Geometry check sheet. Reference: the model listing, model coordinates, mm. A direction names the side the tool comes from. Round coordinates to 2 decimals unless told otherwise and drop trailing zeros. Write each loop counter-clockwise with the first axis right and the second up, starting at its lowest first coordinate (ties: lowest second). Pieces come first, ordered by that corner, then holes. Notation, with made-up numbers: (27, 79) - (41, 79) arc R26 cw to (41, 99) - close; hole circle Ø9 at (-12.5, 47.5). An arc over 180 degrees is marked (long way). Return JSON: item names as keys, results as strings.
```python
from build123d import *

# Parameters (mm, degrees)
BODY_PROFILE_SKETCH_R       = 3
PUMP_BODY_40MM_DEPTH        = 40
BODY_EDGE_FILLET_R8_R       = 8
CSK_HOLE_10_D               = 10
CSK_HOLE_10_CSINK_D         = 12
CSK_HOLE_10_CSINK_ANGLE     = 82
MOUNTING_FLANGE_10MM_DEPTH  = 10
FLANGE_RELIEF_CUT_REACH     = 90.436
FLANGE_RELIEF_CUT_SKETCH_R  = 8
CBORE_HOLE_6_D              = 6
CBORE_HOLE_6_CBORE_D        = 10
CBORE_HOLE_6_CBORE_DEPTH    = 5
SKETCH16_W                  = 3
SKETCH16_H                  = 10
PLAIN_HOLE_6_X10_AT_2_COUNT = 2
PLAIN_HOLE_6_X10_AT_2_PITCH = 80
LOCATING_BOSS_SKETCH_R      = 6
LOCATING_BOSS_12MM_DEPTH    = 12


with BuildPart() as part:
    # Body Profile Sketch → Pump Body 40mm (new body)
    with BuildSketch(Plane(origin=(0, 0, 0), x_dir=(0, 0, -1), z_dir=(1, 0, 0))):
        with BuildLine():
            Line((-12.5, -15.288884851), (-12.5, -36))
            ThreePointArc((-12.5, -36), (-12.104388127, -39.213597032), (-10.941176471, -42.235294118))
            ThreePointArc((-10.941176471, -42.235294118), (-11.140056594, -50.115966043), (-18, -54))
            Line((-18, -54), (-35, -54))
            Line((-35, -54), (-35, -64))
            Line((-35, -64), (35, -64))
            Line((35, -64), (35, -54))
            Line((35, -54), (18, -54))
            ThreePointArc((18, -54), (11.140056594, -50.115966043), (10.941176471, -42.235294118))
            ThreePointArc((10.941176471, -42.235294118), (12.104388127, -39.213597032), (12.5, -36))
            Line((12.5, -36), (12.5, -15.288884851))
            ThreePointArc((12.5, -15.288884851), (12.854205105, -13.25787525), (13.875, -11.466663639))
            ThreePointArc((13.875, -11.466663639), (17.99141486, -0.555869896), (14.556416913, 10.588235294))
            Line((14.556416913, 10.588235294), (6.469518628, 21.705882353))
            ThreePointArc((6.469518628, 21.705882353), (0, 25), (-6.469518628, 21.705882353))
            Line((-6.469518628, 21.705882353), (-14.556416913, 10.588235294))
            ThreePointArc((-14.556416913, 10.588235294), (-17.99141486, -0.555869896), (-13.875, -11.466663639))
            ThreePointArc((-13.875, -11.466663639), (-12.854205105, -13.25787525), (-12.5, -15.288884851))
        make_face()
        with Locations((0, -18)):
            Circle(BODY_PROFILE_SKETCH_R, mode=Mode.SUBTRACT)
        with Locations((0, 18)):
            Circle(BODY_PROFILE_SKETCH_R, mode=Mode.SUBTRACT)
    extrude(amount=PUMP_BODY_40MM_DEPTH)

    # Body Edge Fillet R8
    body_edge_fillet_r8_edges = [part.edges().sort_by_distance(p)[0] for p in [
        (0, -59, -35),
        (0, -59, 35),
        (40, -59, 35),
        (40, -59, -35),
    ]]
    fillet(body_edge_fillet_r8_edges, radius=BODY_EDGE_FILLET_R8_R)

    # Csk Hole Ø10 (through all)
    with Locations(Plane(origin=(10, -54, 27), x_dir=(0, 0, 1), z_dir=(0, 1, 0))):
        with Locations((0, 0), (0, 20)):
            csk_hole_10 = CounterSinkHole(CSK_HOLE_10_D / 2, CSK_HOLE_10_CSINK_D / 2, counter_sink_angle=CSK_HOLE_10_CSINK_ANGLE)

    # Csk Hole Ø10 Mirror: Csk Hole Ø10 across plane
    add(csk_hole_10.mirror(Plane.XY), mode=Mode.SUBTRACT)

    # Sketch7 → Main Bore Ø20 Csk Both Ends (revolve, cut)
    with BuildSketch(Plane(origin=(40, 0, 0), x_dir=(0, 0, -1), z_dir=(0, 1, 0))):
        Polygon((0, 0), (0, 40), (12, 40), (10, 37.699263186), (10, 2.300736814), (12, 0), align=None)
    revolve(axis=Axis((46.35, 0, 0), (-1, 0, 0)), mode=Mode.SUBTRACT)

    # Mounting Flange Sketch → Mounting Flange 10mm (add)
    with BuildSketch(Plane.ZY):
        with BuildLine():
            Line((32, 0), (32, -30))
            ThreePointArc((32, -30), (0, -62), (-32, -30))
            Line((-32, -30), (-32, 0))
            ThreePointArc((-32, 0), (0, 32), (32, 0))
        make_face()
    extrude(amount=MOUNTING_FLANGE_10MM_DEPTH)

    # Flange Relief Cut Sketch → Flange Relief Cut (cut, up to next)
    with BuildSketch(Plane.ZY.offset(10), mode=Mode.PRIVATE) as flange_relief_cut_sk1:
        Circle(FLANGE_RELIEF_CUT_SKETCH_R)
    flange_relief_cut_tool1 = extrude(flange_relief_cut_sk1.sketch, amount=-FLANGE_RELIEF_CUT_REACH, mode=Mode.PRIVATE) & part.part
    add(flange_relief_cut_tool1.solids().sort_by_distance((-10, 0, 0))[0], mode=Mode.SUBTRACT)

    # Sketch9 → Flange Csk Hole Ø18 (revolve, cut)
    with BuildSketch(Plane(origin=(-10, -36, 0), x_dir=(0, 0, 1), z_dir=(0, 1, 0))):
        Polygon((0, 0), (0, 9.797958971), (9, 9.797958971), (9, 2.300736814), (11, 0), align=None)
    revolve(axis=Axis((-16.445314094, -36, 0), (1, 0, 0)), mode=Mode.SUBTRACT)

    # CBore Hole Ø6 (through all)
    with Locations(Plane(origin=(0, -30, -25), x_dir=(0, 0, 1), z_dir=(1, 0, 0))):
        with Locations((0, 0), (0, -30), (50, 0), (50, -30)):
            CounterBoreHole(CBORE_HOLE_6_D / 2, CBORE_HOLE_6_CBORE_D / 2, CBORE_HOLE_6_CBORE_DEPTH)

    # Sketch16 → Plain Hole Ø6 x10 (revolve, cut)
    with BuildSketch(Plane(origin=(0, -55, 0), x_dir=(0, 0, -1), z_dir=(0, 1, 0))):
        with Locations((1.5, 5)):
            Rectangle(SKETCH16_W, SKETCH16_H)
    plain_hole_6_x10 = revolve(axis=Axis((-110, -55, 0), (1, 0, 0)), mode=Mode.SUBTRACT)

    # Plain Hole Ø6 x10 at 2: Plain Hole Ø6 x10 ×2
    with Locations(*[(0, i * PLAIN_HOLE_6_X10_AT_2_PITCH, 0) for i in range(1, PLAIN_HOLE_6_X10_AT_2_COUNT)]):
        add(plain_hole_6_x10, mode=Mode.SUBTRACT)

    # Locating Boss Sketch → Locating Boss 12mm (add)
    with BuildSketch(Plane(origin=(0, 0, 0), x_dir=(0, 0, -1), z_dir=(1, 0, 0))):
        with Locations((0, 25)):
            Circle(LOCATING_BOSS_SKETCH_R)
    extrude(amount=LOCATING_BOSS_12MM_DEPTH)


solid = part.part
```
(1) Material ranges on line 1 along Z through (x, y) = (30, -60); line 2 along Y through (x, z) = (-5.25, 0); line 3 along Y through (x, z) = (23, 0), recorded low to high. Write a range as [from, to].
Response values:
{"line 1": "z = [-35, -32], [-22, 22], [32, 35]", "line 2": "y = [-62, -58], [-52, -45], [-27, -8], [8, 22], [28, 32]", "line 3": "y = [-64, -21], [-15, -10], [10, 15], [21, 25]"}
(2) Section check B-B, the plane z = 16. Enter the section's corners in (x, y), plus the area to 3 significant figures.
Response values:
{"outline": "(-10, -57.71) - (0, -57.71) - (0, -64) - (40, -64) - (40, -53.75) - (0, -53.75) - (0, -8.25) - (40, -8.25) - (40, 8.25) - (0, 8.25) - (0, 27.71) - (-10, 27.71) - close", "area": "1,920 mm^2"}
(3) Gauge pin test, flat ends, axial feed: pin 1 (3 mm diameter, centred on y = -2.5, z = 23.5, fed in from +X); pin 2 (5 mm diameter, centred on x = 23.5, z = -26, fed in from +Y); pin 3 (12 mm diameter, centred on y = -0.5, z = -4, fed in from +X). Record the tip position at first contact, or that the pin passes through.
Response values:
{"pin 1": "stops at x = -5", "pin 2": "stops at y = -54", "pin 3": "stops at x = 37.74"}
(4) Section check C-C, the plane x = 10. Give the number of separate pieces and of enclosed holes in the cut face, plus the area to 3 significant figures.
Response values:
{"separate pieces": "3", "enclosed holes": "3", "area": "2,240 mm^2"}
(5) Access from +Z, -Z, +X, -X, +Y, -Y to the whole of each face (thin tool, end or side, straight path). Record for faces 4 (the face through (20, -26, -12.5)), 5 (the face through (-5, -52, 0)), 6 (the face through (19.72, -39.169, 12.115)), 7 (the face through (-2, -30, -30)).
Response values:
{"face 4": "-Z, +X", "face 5": "-X", "face 6": "+Z, +X", "face 7": "+X"}
(6) Section check A-A, the plane x = 22. Enter the section's corners in (y, z) (3 decimals), plus the area to 3 significant figures.
Response values:
{"outline": "(-64, -35) - (-54, -35) - (-54, -18) arc R8 cw to (-42.235, -10.941) arc R13.25 ccw to (-36, -12.5) - (-15.289, -12.5) arc R6 cw to (-11.467, -13.875) arc R18 ccw to (10.588, -14.556) - (21.706, -6.47) arc R8 ccw to (21.706, 6.47) - (10.588, 14.556) arc R18 ccw to (-11.467, 13.875) arc R6 cw to (-15.289, 12.5) - (-36, 12.5) arc R13.25 ccw to (-42.235, 10.941) arc R8 cw to (-54, 18) - (-54, 35) - (-64, 35) - close; hole circle Ø6 at (-18, 0); hole circle Ø20 at (0, 0); hole circle Ø6 at (18, 0)", "area": "2,360 mm^2"}
(7) Release check for a two-part mould opening along X. For faces 1 (the face through (19.72, -50.017, 11.081)), 2 (the face through (13, -60, -31)), 3 (the face through (0, 25, 0)) record: pulls with the +X half, pulls with the -X half, needs draft (parallel to the pull), parting line crosses it, or undercut.
Response values:
{"face 1": "needs draft", "face 2": "undercut", "face 3": "pulls with the -X half"}
